from build123d import *

# Parameters (mm, degrees)
EXTRUDE_365_DEPTH = 12.5
SKETCH_4_W        = 0.8
SKETCH_4_H        = 12.320508076
CHAMFER_2074_SIZE = 2
FILLET_2128_R     = 0.8


with BuildPart() as part:
    # 草图1 → Extrude 365 (new body)
    with BuildSketch(Plane(origin=(0, 0, 0), x_dir=(0, 0, -1), z_dir=(1, 0, 0))):
        Polygon((15, 8.660254038), (15, -8.660254038), (0, -17.320508076), (-15, -8.660254038), (-15, 8.660254038), (0, 17.320508076), align=None)
    extrude(amount=EXTRUDE_365_DEPTH)

    # 草图2 → 凸台-旋转1 (revolve)
    with BuildSketch(Plane.XY, mode=Mode.PRIVATE) as revolve_1_sk:
        Polygon((0, 0), (102.5, 0), (102.5, 7.835), (102.5, 10), (7.791693541, 10), (0, 10), align=None)
    revolve(revolve_1_sk.sketch.rotate(Axis((0, 0, 0), (1, 0, 0)), 90), axis=Axis((0, 0, 0), (1, 0, 0)))

    # 草图3 → 切除-旋转1 (revolve, cut)
    with BuildSketch(Plane.XY):
        Polygon((0, 15), (4.226497308, 22.320508076), (4.226497308, 27.320508076), (-10, 27.320508076), (-10, 15), align=None)
    revolve(axis=Axis((0, 0, 0), (1, 0, 0)), mode=Mode.SUBTRACT)

    # 草图5 → 切除-旋转2 (revolve, cut)
    with BuildSketch(Plane.XY):
        Polygon((12.5, 15), (8.273502692, 22.320508076), (8.273502692, 27.320508076), (18.273502692, 27.320508076), (18.273502692, 15), align=None)
    revolve(axis=Axis((0, 0, 0), (1, 0, 0)), mode=Mode.SUBTRACT)

    # 草图4 → 切除-旋转3 (revolve, cut)
    with BuildSketch(Plane.XY, mode=Mode.PRIVATE) as cut_revolve_3_sk:
        with Locations((12.1, 21.160254038)):
            Rectangle(SKETCH_4_W, SKETCH_4_H)
    revolve(cut_revolve_3_sk.sketch.rotate(Axis((0, 0, 0), (1, 0, 0)), 270), axis=Axis((0, 0, 0), (1, 0, 0)), mode=Mode.SUBTRACT)

    # Chamfer 2074
    chamfer_2074_edges = [part.edges().sort_by_distance(p)[0] for p in [
        (102.5, 0, -10),
    ]]
    chamfer(chamfer_2074_edges, length=CHAMFER_2074_SIZE)

    # Fillet 2128
    fillet_2128_edges = [part.edges().sort_by_distance(p)[0] for p in [
        (12.5, 0, -10),
    ]]
    fillet(fillet_2128_edges, radius=FILLET_2128_R)


solid = part.part
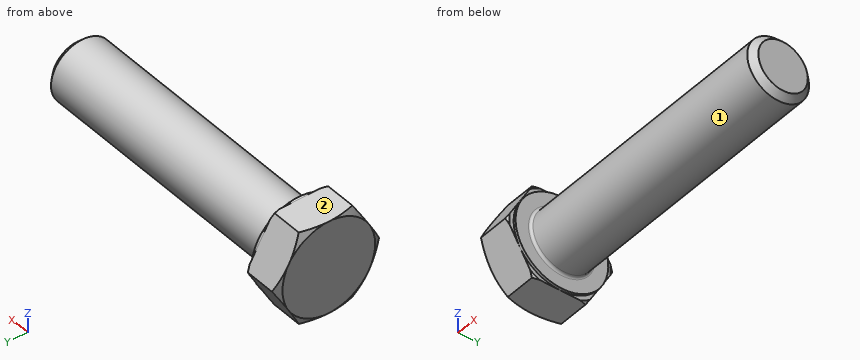
The model under review builds one solid part; all positions refer to its coordinate system, in mm. Face numbers are marked on the shaded views. A direction names the side the tool comes from. Round coordinates to 2 decimals unless told otherwise and drop trailing zeros. Loops run counter-clockwise (first coordinate to the right, second up) from the corner with the lowest first, then second, coordinate; pieces in that order, holes last. Notation, with made-up numbers: (56.5, 52.25) -> (106.5, 52.25) arc R22 cw to (106.5, 68.25) -> close; hole circle Ø9 at (48, 23.5). An arc over 180 degrees is marked (long way). Write item = value, one per line. Start each with the question number.
Item 1: Take a section at A-A on x = 85. Give the boundary of the cut face in (y, z), plus the area to 3 significant figures.
Item 2: Insertion check: pin 1 (3 mm diameter, centred on y = -12, z = 4, fed in from +X); pin 2 (5 mm diameter, centred on x = 45.5, z = -5.5, fed in from +Y); pin 3 (6 mm diameter, centred on x = 59.5, z = 5, fed in from -Y). Each pin has a flat end and moves straight along its axis. Give the tip position at first contact, or say it passes through.
Item 3: To check wall thickness, follow L1, parallel to X at y = 13, z = -5.5; L2, parallel to Y at x = 33, z = 0; L3, parallel to Y at x = 34, z = -5. State the ranges of each line that lie inside material, in increasing order.
Item 4: For the marked faces 1 and 2, list the 3-axis set-ups (+Z, -Z, +X, -X, +Y, -Y) from which the entire face can be reached by the end or side of a thin tool; tool diameter is ignored.
Result:
q1.outline = circle Ø20 at (0, 0)
q1.area = 314 mm²
q2.pin_1 = 12.5
q2.pin_2 = 9.54
q2.pin_3 = -9.8
q3.L1 = 0 to 12.5
q3.L2 = -10 to 10
q3.L3 = -8.66 to 8.66
q4.face_1 = +X
q4.face_2 = +Z, +X, -X, +Y, -Y
